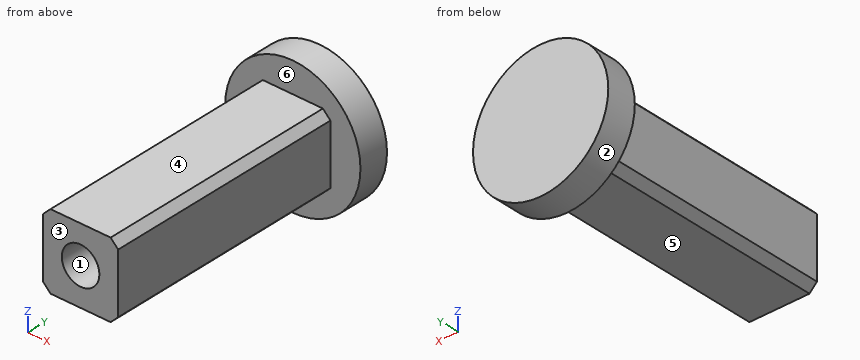
from build123d import *

# Parameters (mm, degrees)
SKETCH_1_R             = 4.5
EXTRUDE_1_DEPTH        = 9
CUT_EXTRUDE_START      = -16
SKETCH_2_R             = 4.5
SKETCH_2_W             = 5
SKETCH_2_H             = 5
CUT_EXTRUDE_1_DEPTH    = 16
HOLE_WIZARD_M3_1_D     = 2.5
HOLE_WIZARD_M3_1_DEPTH = 8.5
HOLE_WIZARD_M3_1_TIP   = 0.751075774
CHAMFER_1_SIZE         = 0.5


with BuildPart() as part:
    # 草图1 → 凸台-拉伸1 (new, symmetric)
    with BuildSketch(Plane(origin=(0, 0, 0), x_dir=(1, 0, 0), z_dir=(0, 1, 0))):
        with Locations(Location((0, 0, 0), (0, 0, 270))):
            Circle(SKETCH_1_R)
    extrude(amount=EXTRUDE_1_DEPTH, both=True)

    # 草图2 → 切除-拉伸1 (cut)
    with BuildSketch(Plane.XZ.offset(9).offset(CUT_EXTRUDE_START)):
        with Locations(Location((0, 0, 0), (0, 0, 270))):
            Circle(SKETCH_2_R)
        Rectangle(SKETCH_2_W, SKETCH_2_H, mode=Mode.SUBTRACT)
    extrude(amount=CUT_EXTRUDE_1_DEPTH, mode=Mode.SUBTRACT)

    # M3 螺纹孔1
    with Locations(Plane(origin=(0, -9, 0), x_dir=(-1, 0, 0), z_dir=(0, -1, 0))):
        with Locations((0, 0)):
            Hole(HOLE_WIZARD_M3_1_D / 2, depth=HOLE_WIZARD_M3_1_DEPTH)
            with Locations((0, 0, -(HOLE_WIZARD_M3_1_DEPTH + HOLE_WIZARD_M3_1_TIP / 2))):  # 118° drill point
                Cone(0, HOLE_WIZARD_M3_1_D / 2, HOLE_WIZARD_M3_1_TIP, mode=Mode.SUBTRACT)

    # 倒角1
    chamfer_1_edges = [part.edges().sort_by_distance(p)[0] for p in [
        (2.5, -1, -2.5),
        (-2.5, -1, -2.5),
        (-2.5, -1, 2.5),
        (2.5, -1, 2.5),
    ]]
    chamfer(chamfer_1_edges, length=CHAMFER_1_SIZE)


solid = part.part
Read the model definition and answer for the solid it produces. Units are mm, in the model's axes. Face numbers are marked on the shaded views. A direction names the side the tool comes from. Give positions to 0.01 mm unless a question says otherwise; leave off trailing zeros. Loops run counter-clockwise (first coordinate to the right, second up) from the corner with the lowest first, then second, coordinate; pieces in that order, holes last. Notation, with made-up numbers: (84.5, 25.5) -> (121.5, 25.5) arc R10 cw to (121.5, 38.5) -> close; hole circle Ø5 at (67, -30). An arc over 180 degrees is marked (long way). Use a Markdown table: item, result.
Q1. Find the intervals of material crossed by line 1 along Z through (x, y) = (0, -4); line 2 along Y through (x, z) = (-3.25, 0.5); line 3 along Z through (x, y) = (0.5, -1), in increasing order.
Solved:
| item | result |
|---|---|
| line 1 | z = -2.5 to -1.25, 1.25 to 2.5 |
| line 2 | y = 7 to 9 |
| line 3 | z = -2.5 to -1.15, 1.15 to 2.5 |
Q2. Section C-C, the plane z = -2.75 is taken. Determine the outline of the cut face in (x, y).
Solved:
| item | result |
|---|---|
| outline | (-3.56, 7) -> (3.56, 7) -> (3.56, 9) -> (-3.56, 9) -> close |
Q3. Each of these flat-tipped pins is pushed along its axis until it touches: pin 1 (1.5 mm diameter, centred on x = -0.5, y = -5.5, fed in from +Z); pin 2 (4.5 mm diameter, centred on x = 0, y = -0.5, fed in from -Z); pin 3 (4.5 mm diameter, centred on y = 3, z = -1, fed in from -X); pin 4 (3 mm diameter, centred on y = 6, z = 1, fed in from -X). Where does it stop, or does it pass through?
Solved:
| item | result |
|---|---|
| pin 1 | stops at z = 2.5 |
| pin 2 | stops at z = -2.5 |
| pin 3 | stops at x = -2.5 |
| pin 4 | stops at x = -4.5 |
Q4. A tool of negligible diameter and unlimited length cuts with its end or side. For the marked faces 4, 5 and 6, from which of +Z, -Z, +X, -X, +Y, -Y can it reach the whole face along a straight path? Write none if from no direction.
Solved:
| item | result |
|---|---|
| face 4 | +Z, +X, -X, -Y |
| face 5 | -Z, +X, -X, -Y |
| face 6 | -Y |
Q5. Section B-B, the plane y = 7.75 is taken. Determine the outline of the cut face in (x, z), then the cut area to 3 significant figures.
Solved:
| item | result |
|---|---|
| outline | circle Ø9 at (0, 0) |
| area | 63.6 mm^2 |
Q6. Determine the mould class of the marked faces 1, 2 and 3 for opening direction X: pulls with the +X half, pulls with the -X half, needs draft (parallel to the pull), parting line crosses it, or undercut.
Solved:
| item | result |
|---|---|
| face 1 | undercut |
| face 2 | parting line crosses it |
| face 3 | needs draft |
Q7. Section A-A, the plane y = -7 is taken. Determine the outline of the cut face in (x, z), then the cut area to 3 significant figures.
Solved:
| item | result |
|---|---|
| outline | (-2.5, -2) -> (-2, -2.5) -> (2, -2.5) -> (2.5, -2) -> (2.5, 2) -> (2, 2.5) -> (-2, 2.5) -> (-2.5, 2) -> close; hole circle Ø2.5 at (0, 0) |
| area | 19.6 mm^2 |
